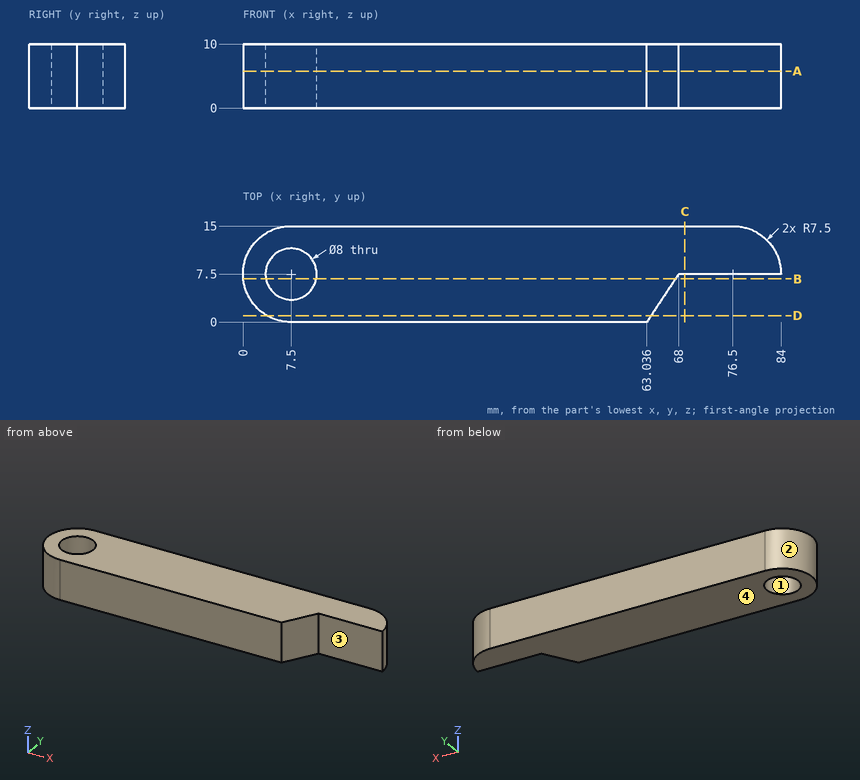
Source: three-view drawing plus pictorial views. Frame: mm from the lowest corner of the part. Round coordinates to 2 decimals unless told otherwise and drop trailing zeros. Order: outer loops, then holes, each group sorted by start corner. A loop starts at its lowest first (then second) coordinate and runs counter-clockwise, first axis right, second up. Notation, with made-up numbers: M 33,73 L 43,73 A15 cw 43,91 Z; hole C 69,58 d11. An arc over 180 degrees is marked long. One line per item, written item: value.
(1) Cut plane A-A (z = 5.75). Return the cut outline in (x, y) (1 decimal), and give its area (4 significant figures).
Result sheet:
outline: M 7.5,0 L 63,0 L 68,7.5 L 84,7.5 A7.5 ccw 76.5,15 L 7.5,15 A7.5 ccw Z; hole C 7.5,7.5 d8
area: 1,035 mm2
(2) Cut plane B-B (y = 6.75). Return the cut outline in (x, z), and give its area (3 significant figures).
Result sheet:
outline: M 0.04,0 L 3.57,0 L 3.57,10 L 0.04,10 Z; M 11.43,0 L 67.5,0 L 67.5,10 L 11.43,10 Z
area: 596 mm2
(3) Cut plane D-D (y = 1). Return the cut outline in (x, z), and give its area (3 significant figures).
Result sheet:
outline: M 3.76,0 L 63.7,0 L 63.7,10 L 3.76,10 Z
area: 599 mm2
(4) Pull-direction query (Y, two-part tool) for the marked faces 1, 2, 3 and 4; classes: pulls with the +Y half, pulls with the -Y half, needs draft (parallel to the pull), parting line crosses it, or undercut.
Result sheet:
face 1: undercut
face 2: parting line crosses it
face 3: pulls with the -Y half
face 4: needs draft
(5) Pin query (flat end, axial travel): P1, Ø2, axis at y = 3, z = 4, coming from the -X side. Return the tip coordinate at first contact, or that it passes through.
Result sheet:
P1: x = 0.87
(6) Cut plane C-C (x = 69). Return the cut outline in (y, z).
Result sheet:
outline: M 7.5,0 L 15,0 L 15,10 L 7.5,10 Z
(7) Line query: probe 1 along Y at (x, z) = (7.5, 7); probe 2 along X at (y, z) = (9, 9.5); probe 3 along Y at (x, z) = (69.5, 2.25). Output: solid intervals per line, ascending. Write a range as [from, to].
Result sheet:
probe 1: [0, 3.5], [11.5, 15]
probe 2: [0.15, 3.79], [11.21, 83.85]
probe 3: [7.5, 15]
